Design review of the part built by this model. Coordinates are the model's own, in mm. Round coordinates to 2 decimals unless told otherwise and drop trailing zeros. Loops run counter-clockwise (first coordinate to the right, second up) from the corner with the lowest first, then second, coordinate; pieces in that order, holes last. Notation, with made-up numbers: (43.25, 7) - (93.25, 7) arc R20 ccw to (93.25, 36) - close; hole circle Ø7 at (52.25, 70.5). An arc over 180 degrees is marked (long way). Return JSON: item names as keys, results as strings. Group by question number.
(1) We need section A-A, the plane x = 0. Write out the cut boundary in (y, z), and give its area (3 significant figures).
(2) Clearance check with a flat-ended pin moving along its axis: pin 1 (2 mm diameter, centred on x = 0, z = 50, fed in from +Y). State where the tip first meets the part, or that it passes through.
(3) Wall thickness on L1, parallel to X at y = -0.6, z = 50; L2, parallel to Z at x = -0.5, y = -1.45; L3, parallel to Z at x = 0.65, y = 0.75: over which ranges is each line inside the solid? List them lowest first. Write a range as [from, to].
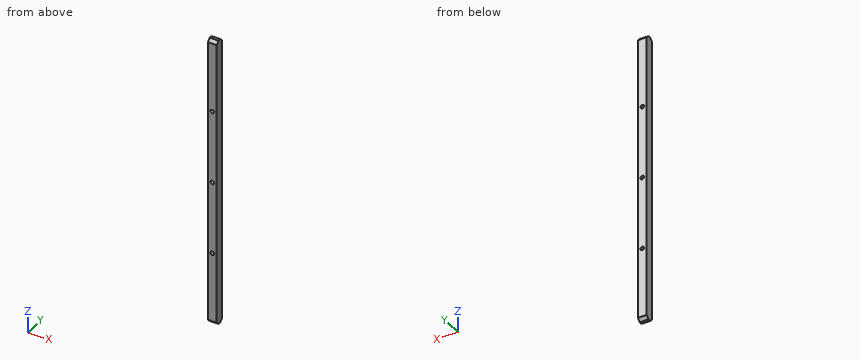
from build123d import *

# Parameters (mm, degrees)
SKETCH_1_W         = 6
SKETCH_1_H         = 6
EXTRUDE_1_DEPTH    = 200
HOLE_WIZARD_M3_1_D = 2.5
CHAMFER_1_SIZE     = 2


with BuildPart() as part:
    # 草图1 → 凸台-拉伸1 (new body)
    with BuildSketch(Plane.XY):
        Rectangle(SKETCH_1_W, SKETCH_1_H)
    extrude(amount=EXTRUDE_1_DEPTH)

    # M3 螺纹孔1 (through all)
    with Locations(Plane(origin=(0, 3, 50), x_dir=(0, 0, 1), z_dir=(0, 1, 0))):
        with Locations((0, 0), (50, 0), (100, 0)):
            Hole(HOLE_WIZARD_M3_1_D / 2)

    # 倒角1
    chamfer_1_edges = [part.edges().sort_by_distance(p)[0] for p in [
        (0, -3, 200),
        (0, -3, 0),
        (0, 3, 0),
        (0, 3, 200),
    ]]
    chamfer(chamfer_1_edges, length=CHAMFER_1_SIZE)


solid = part.part
Solutions:
{
 "1": {"outline": "(-3, 2) - (-1, 0) - (1, 0) - (3, 2) - (3, 48.75) - (-3, 48.75) - close; (-3, 51.25) - (3, 51.25) - (3, 98.75) - (-3, 98.75) - close; (-3, 101.25) - (3, 101.25) - (3, 148.75) - (-3, 148.75) - close; (-3, 151.25) - (3, 151.25) - (3, 198) - (1, 200) - (-1, 200) - (-3, 198) - close", "area": "1,150 mm^2"},
 "2": {"pin 1": "through"},
 "3": {"L1": "[-3, -1.25], [1.25, 3]", "L2": "[0.45, 48.85], [51.15, 98.85], [101.15, 148.85], [151.15, 199.55]", "L3": "[0, 48.93], [51.07, 98.93], [101.07, 148.93], [151.07, 200]"}
}
